Check sheet for the modelled part. Datum: model origin and axes. Units: mm. A direction names the side the tool comes from. Give positions to 0.01 mm unless a question says otherwise; leave off trailing zeros. Loops run counter-clockwise (first coordinate to the right, second up) from the corner with the lowest first, then second, coordinate; pieces in that order, holes last. Notation, with made-up numbers: (11.5, 61.25) - (59.5, 61.25) arc R24 ccw to (59.5, 86.25) - close; hole circle Ø2 at (55.5, 45). An arc over 180 degrees is marked (long way). Use one line per item in the form item = value.
from build123d import *

# Parameters (mm, degrees)
SKETCH2_OUTSIDE_W   = 68.656
SKETCH2_OUTSIDE_H   = 68.656
SKETCH2_OUTSIDE_W_2 = 34
SKETCH2_OUTSIDE_H_2 = 45
CUT_EXTRUDE1_DEPTH  = 43.731721238
SKETCH3_R           = 5.5
CUT_EXTRUDE2_DEPTH  = 53.261362401
M4_TAPPED_HOLE1_D   = 3.3
SKETCH14_R          = 2
CUT_EXTRUDE5_DEPTH  = 38.030392923
CHAMFER1_SIZE       = 0.5
CHAMFER2_SIZE       = 0.5
CUT_EXTRUDE6_DEPTH  = 52.829045911


with BuildPart() as part:
    # Sketch1 → Revolve1 (revolve)
    with BuildSketch(Plane(origin=(0, 0, 0), x_dir=(0, 0, -1), z_dir=(1, 0, 0)), mode=Mode.PRIVATE) as revolve1_sk:
        Polygon((0, -12), (11, -12), (11, 0), (25, 0), (25, 12), (17, 12), (17, 14), (12.5, 14), (12.5, 29), (12, 29), (12, 30.3), (12.5, 30.3), (12.5, 32), (0, 32), align=None)
    revolve(revolve1_sk.sketch.rotate(Axis((0, 78.762169225, 0), (0, -1, 0)), 180), axis=Axis((0, 78.762169225, 0), (0, -1, 0)))

    # Sketch2 outside → Cut-Extrude1 (cut, through all)
    with BuildSketch(Plane(origin=(0, 12, 0), x_dir=(1, 0, 0), z_dir=(0, 1, 0))):
        Rectangle(SKETCH2_OUTSIDE_W, SKETCH2_OUTSIDE_H)
        Rectangle(SKETCH2_OUTSIDE_W_2, SKETCH2_OUTSIDE_H_2, mode=Mode.SUBTRACT)
    extrude(amount=-CUT_EXTRUDE1_DEPTH, mode=Mode.SUBTRACT)

    # Sketch3 → Cut-Extrude2 (cut, through all)
    with BuildSketch(Plane.XZ.offset(12)):
        with Locations(Location((0, 0, 0), (0, 0, 270))):
            Circle(SKETCH3_R)
    extrude(amount=-CUT_EXTRUDE2_DEPTH, mode=Mode.SUBTRACT)

    # M4 Tapped Hole1 (through all)
    with Locations(Plane(origin=(0, 0, 0), x_dir=(-1, 0, 0), z_dir=(0, -1, 0))):
        with Locations((-12.5, 17.5), (12.5, -17.5)):
            Hole(M4_TAPPED_HOLE1_D / 2)

    # Sketch14 → Cut-Extrude5 (cut, through all)
    with BuildSketch(Plane(origin=(0, 12, 0), x_dir=(1, 0, 0), z_dir=(0, 1, 0))):
        with Locations(Location((12.5, -17.5, 0), (0, 0, 270))):
            Circle(SKETCH14_R)
        with Locations(Location((-12.5, 17.5, 0), (0, 0, 270))):
            Circle(SKETCH14_R)
    extrude(amount=-CUT_EXTRUDE5_DEPTH, mode=Mode.SUBTRACT)

    # Chamfer1
    chamfer1_edges = [part.edges().sort_by_distance(p)[0] for p in [
        (0, -12, -11),
        (0, 32, -12.5),
    ]]
    chamfer(chamfer1_edges, length=CHAMFER1_SIZE)

    # Chamfer2
    chamfer2_edges = [part.edges().sort_by_distance(p)[0] for p in [
        (0, 32, 5.5),
        (0, -12, 5.5),
    ]]
    chamfer(chamfer2_edges, length=CHAMFER2_SIZE)

    # Sketch15 → Cut-Extrude6 (cut, through all)
    with BuildSketch(Plane(origin=(17, 0, 0), x_dir=(0, 0, -1), z_dir=(1, 0, 0))):
        with BuildLine():
            Line((-3, 9), (3, 9))
            ThreePointArc((3, 9), (6, 6), (3, 3))
            Line((3, 3), (-3, 3))
            ThreePointArc((-3, 3), (-6, 6), (-3, 9))
        make_face()
    extrude(amount=-CUT_EXTRUDE6_DEPTH, mode=Mode.SUBTRACT)


solid = part.part
Item 1: Gauge pin test, flat ends, axial feed: P1, Ø10, axis at x = -2.5, z = -4.5, coming from the +Y side; P2, Ø4.5, axis at x = -12.5, z = 17.5, coming from the -Y side; P3, Ø10, axis at x = 0, z = 0, coming from the +Y side; P4, Ø10, axis at x = -12.5, y = 20, coming from the +Z side. Record the tip position at first contact, or that the pin passes through.
Answer block:
P1 = 32
P2 = 0
P3 = through
P4 = 10
Item 2: Section check B-B on y = 25.5. Record the boundary of the cut face in (x, z).
Answer block:
outline = circle Ø25 at (0, 0); hole circle Ø11 at (0, 0)
Item 3: Thickness scan on L1, parallel to X at y = 6.25, z = -17.5; L2, parallel to Y at x = -14.5, z = -8; L3, parallel to Y at x = -8, z = -5.5. Record the ranges inside material, lowest first.
Answer block:
L1 = -17 to -14.5, -10.5 to 10.85, 14.15 to 17
L2 = 0 to 14
L3 = -12 to 4.34, 7.66 to 32
Item 4: Mould release check, pull along Y, two halves, no side actions. Record for faces 4 (the face through (-9, 14, -9)), 5 (the face through (0.242, 19.412, 5.495)), 6 (the face through (-10, 30.3, 7)): released by +Y, released by -Y, zero draft, split by the parting line, or undercut.
Answer block:
face_4 = released by +Y
face_5 = zero draft
face_6 = undercut
Item 5: Access from +Z, -Z, +X, -X, +Y, -Y to the whole of each face (thin tool, end or side, straight path). Record for faces 1 (the face through (-11, 3, 0)), 2 (the face through (-3.755, 21.605, 11.923)), 3 (the face through (-1, 12, -18)).
Answer block:
face_1 = +X, -X
face_2 = +Y
face_3 = -Z, +Y
Item 6: Section check C-C on z = -2. Give the number of separate pieces and of enclosed holes in the cut face, then the cut area to 3 significant figures.
Answer block:
separate_pieces = 4
enclosed_holes = 0
area = 584 mm2
Item 7: Section check A-A on y = 6. Record the boundary of the cut face in (x, z).
Answer block:
outline = (-17, -18.33) arc R25 ccw to (-10.9, -22.5) - (10.9, -22.5) arc R25 ccw to (17, -18.33) - (17, -6) - (-17, -6) - close; (-17, 6) - (17, 6) - (17, 18.33) arc R25 ccw to (10.9, 22.5) - (-10.9, 22.5) arc R25 ccw to (-17, 18.33) - close; hole circle Ø4 at (-12.5, -17.5); hole circle Ø3.3 at (-12.5, 17.5); hole circle Ø4 at (12.5, 17.5); hole circle Ø3.3 at (12.5, -17.5)
